The model under review builds one solid part; all positions refer to its coordinate system, in mm. Face numbers are marked on the shaded views. A direction names the side the tool comes from. Coordinates: 2 decimals unless noted, no trailing zeros. Write each loop counter-clockwise with the first axis right and the second up, starting at its lowest first coordinate (ties: lowest second). Pieces come first, ordered by that corner, then holes.
1) Add section D-D, the plane z = 78.5. State the section outline as (x, y) points.
2) For P1, Ø1, axis at y = -95.5, z = 317.5, coming from the -X side; P2, Ø5, axis at y = -160.5, z = 350, coming from the -X side; P3, Ø12, axis at x = -647, z = 261, coming from the +Y side, all flat-tipped, find the tip position at first contact; note any pin that passes through.
3) For line 1 (X direction, y = -90, z = 228.5); line 2 (Y direction, x = -600.5, z = 94); line 3 (Y direction, x = -598, z = 358), list the stretches that pass through material, from the lowest coordinate up.
4) Add section B-B, the plane z = 302. State the section outline as (x, y) points.
5) Mouldability with a two-part tool opening along X and no side actions: class the marked faces 1, 2 and 3 as released by +X, released by -X, zero draft, split by the parting line, or undercut.
6) Add section A-A, the plane y = -90. State the section outline as (x, z) points, then the cut area to 3 significant figures.
7) Add section C-C, the plane y = -125.5. State the section outline as (x, z) points, then the cut area to 3 significant figures.
8) Machinability: for the marked faces 4 and 5, which of the approach directions +Z, -Z, +X, -X, +Y, -Y give a long, thin tool a straight path to every point of the face, cutting with its end or side? Answer none if there is none.
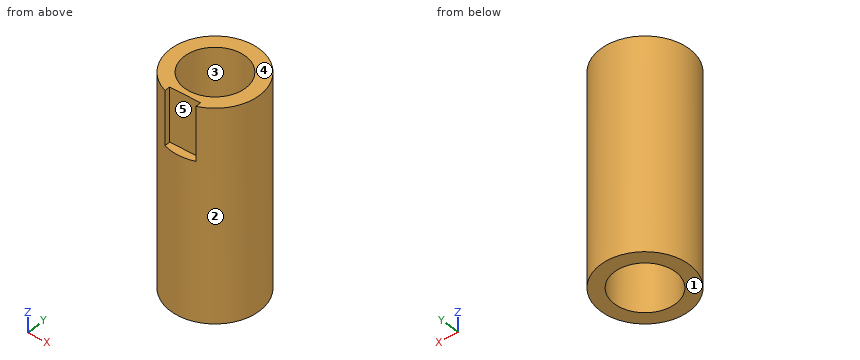
from build123d import *

# Parameters (mm, degrees)
SKETCH1_R               = 80
BOSS_EXTRUDE1_DEPTH     = 380
CUT_EXTRUDE1_START      = -97
CUT_EXTRUDE1_DEPTH      = 97
CUT_EXTRUDE2_DEPTH      = 798.2092078
CUT_EXTRUDE2_DEPTH_BACK = 798.2092078
SKETCH3_R               = 55


with BuildPart() as part:
    # Sketch1 → Boss-Extrude1 (new body)
    with BuildSketch(Plane.XY):
        with Locations((-599.884196758, -90)):
            Circle(SKETCH1_R)
    extrude(amount=BOSS_EXTRUDE1_DEPTH)

    # Sketch2 → Cut-Extrude1 (cut)
    with BuildSketch(Plane.XY.offset(380).offset(CUT_EXTRUDE1_START)):
        with BuildLine():
            ThreePointArc((-627.384196758, -165.124896007), (-599.884196758, -170), (-572.384196758, -165.124896007))
            Line((-572.384196758, -165.124896007), (-572.384196758, -155))
            Line((-572.384196758, -155), (-627.384196758, -155))
            Line((-627.384196758, -155), (-627.384196758, -165.124896007))
        make_face()
    extrude(amount=CUT_EXTRUDE1_DEPTH, mode=Mode.SUBTRACT)

    # Sketch3 → Cut-Extrude2 (cut, two sides: drawn at the far end of the back side and taken through both)
    with BuildSketch(Plane.XY.offset(380).offset(-CUT_EXTRUDE2_DEPTH_BACK)):
        with Locations((-599.884196758, -90)):
            Circle(SKETCH3_R)
    extrude(amount=CUT_EXTRUDE2_DEPTH + CUT_EXTRUDE2_DEPTH_BACK, mode=Mode.SUBTRACT)


solid = part.part
Geometry results:
1. outline: circle Ø160 at (-599.88, -90); hole circle Ø110 at (-599.88, -90)
2. P1: stops at x = -679.73
2. P2: stops at x = -642.03
2. P3: stops at y = -21.37
3. line 1: x = -679.88 to -654.88, -544.88 to -519.88
3. line 2: y = -170 to -145, -35 to -10
3. line 3: y = -155 to -144.97, -35.03 to -10.02
4. outline: (-627.38, -165.12) - (-627.38, -155) - (-572.38, -155) - (-572.38, -165.12) arc R80 ccw (long way) to start; hole circle Ø110 at (-599.88, -90)
5. face 1: zero draft
5. face 2: split by the parting line
5. face 3: undercut
6. outline: (-679.88, 0) - (-654.88, 0) - (-654.88, 380) - (-679.88, 380) - close; (-544.88, 0) - (-519.88, 0) - (-519.88, 380) - (-544.88, 380) - close
6. area: 19,000 mm2
7. outline: (-671.58, 0) - (-641.89, 0) - (-641.89, 380) - (-671.58, 380) - close; (-557.88, 0) - (-528.19, 0) - (-528.19, 380) - (-557.88, 380) - close
7. area: 22,600 mm2
8. face 4: +Z, +X, -X, +Y, -Y
8. face 5: +Z, -Y
